The listing builds one solid part. Answer for the finished solid, in the listing's coordinates (mm). Face numbers are marked on the shaded views. A direction names the side the tool comes from. Give positions to 0.01 mm unless a question says otherwise; leave off trailing zeros. Order: outer loops, then holes, each group sorted by start corner. A loop starts at its lowest first (then second) coordinate and runs counter-clockwise, first axis right, second up. Notation, with made-up numbers: (30, -13.75) - (81, -13.75) arc R20 ccw to (81, 20.25) - close; hole circle Ø4 at (4, 14). An arc over 180 degrees is marked (long way). Answer in a Markdown table with one row per item. Add a question column.
```python
from build123d import *

# Parameters (mm, degrees)
BASE_PLATE_SKETCH_W        = 100
BASE_PLATE_SKETCH_H        = 60
BASE_PLATE_100X60X25_DEPTH = 25
T_BLOCK_SKETCH_W           = 70
T_BLOCK_SKETCH_H           = 40
T_BLOCK_70X40X30_DEPTH     = 30
SLOT_15X20_SKETCH_W        = 15
SLOT_15X20_SKETCH_H        = 20
SLOT_15X20_DEPTH_6_DEPTH   = 6
SECOND_SLOT_SKETCH_W       = 15
SECOND_SLOT_SKETCH_H       = 20
SECOND_SLOT_DEPTH_6_DEPTH  = 6
SIDE_ARC_NOTCH_DEPTH       = 60
END_ARC_NOTCH_DEPTH        = 100
BLOCK_RECESS_A_SKETCH_W    = 26
BLOCK_RECESS_A_SKETCH_H    = 5
BLOCK_RECESS_A_DEPTH       = 30
BLOCK_RECESS_B_SKETCH_W    = 26
BLOCK_RECESS_B_SKETCH_H    = 5
BLOCK_RECESS_B_DEPTH       = 30
CROSS_HOLE_SKETCH_R        = 10
CROSS_HOLE_DEPTH           = 55
WEDGE_CUT_A_DEPTH          = 30
WEDGE_FILL_A_DEPTH         = 10
WEDGE_CUT_B_DEPTH          = 30
WEDGE_FILL_B_DEPTH         = 10


with BuildPart() as part:
    # Base Plate Sketch → Base Plate 100x60x25 (new body)
    with BuildSketch(Plane.XY):
        with Locations((50, -30)):
            Rectangle(BASE_PLATE_SKETCH_W, BASE_PLATE_SKETCH_H)
    extrude(amount=BASE_PLATE_100X60X25_DEPTH)

    # T-Block Sketch → T-Block 70x40x30 (add)
    with BuildSketch(Plane.XY.offset(25)):
        with Locations((50, -30)):
            Rectangle(T_BLOCK_SKETCH_W, T_BLOCK_SKETCH_H)
    extrude(amount=T_BLOCK_70X40X30_DEPTH)

    # Slot 15x20 Sketch → Slot 15x20 Depth 6 (cut)
    with BuildSketch(Plane.XY.offset(25)):
        with Locations((7.5, -30)):
            Rectangle(SLOT_15X20_SKETCH_W, SLOT_15X20_SKETCH_H)
    extrude(amount=-SLOT_15X20_DEPTH_6_DEPTH, mode=Mode.SUBTRACT)

    # Second Slot Sketch → Second Slot Depth 6 (cut)
    with BuildSketch(Plane.XY.offset(25)):
        with Locations((92.5, -30)):
            Rectangle(SECOND_SLOT_SKETCH_W, SECOND_SLOT_SKETCH_H)
    extrude(amount=-SECOND_SLOT_DEPTH_6_DEPTH, mode=Mode.SUBTRACT)

    # Side Arc Notch Sketch → Side Arc Notch (cut)
    with BuildSketch(Plane.XZ.offset(60)):
        with BuildLine():
            Line((30, 0), (70, 0))
            ThreePointArc((70, 0), (50, 20), (30, 0))
        make_face()
    extrude(amount=-SIDE_ARC_NOTCH_DEPTH, mode=Mode.SUBTRACT)

    # End Arc Notch Sketch → End Arc Notch (cut)
    with BuildSketch(Plane.ZY):
        with BuildLine():
            Line((0, -15), (0, -45))
            ThreePointArc((0, -45), (15, -30), (0, -15))
        make_face()
    extrude(amount=-END_ARC_NOTCH_DEPTH, mode=Mode.SUBTRACT)

    # Block Recess A Sketch → Block Recess A (cut)
    with BuildSketch(Plane.XY.offset(55)):
        with Locations((50, -12.5)):
            Rectangle(BLOCK_RECESS_A_SKETCH_W, BLOCK_RECESS_A_SKETCH_H)
    extrude(amount=-BLOCK_RECESS_A_DEPTH, mode=Mode.SUBTRACT)

    # Block Recess B Sketch → Block Recess B (cut)
    with BuildSketch(Plane.XY.offset(55)):
        with Locations((50, -47.5)):
            Rectangle(BLOCK_RECESS_B_SKETCH_W, BLOCK_RECESS_B_SKETCH_H)
    extrude(amount=-BLOCK_RECESS_B_DEPTH, mode=Mode.SUBTRACT)

    # Cross Hole Sketch → Cross Hole (cut)
    with BuildSketch(Plane.XY.offset(55)):
        with Locations((50, -30)):
            Circle(CROSS_HOLE_SKETCH_R)
    extrude(amount=-CROSS_HOLE_DEPTH, mode=Mode.SUBTRACT)

    # Wedge Cut A Sketch → Wedge Cut A (cut)
    with BuildSketch(Plane.XZ.offset(50)):
        Polygon((15, 55), (30, 55), (15, 25), align=None)
    extrude(amount=-WEDGE_CUT_A_DEPTH, mode=Mode.SUBTRACT)

    # Wedge Fill A Sketch → Wedge Fill A (add)
    with BuildSketch(Plane.XZ.offset(50)):
        Polygon((15, 25), (15, 55), (30, 55), align=None)
    extrude(amount=-WEDGE_FILL_A_DEPTH)

    # Wedge Cut B Sketch → Wedge Cut B (cut)
    with BuildSketch(Plane.XZ.offset(50)):
        Polygon((85, 55), (70, 55), (85, 25), align=None)
    extrude(amount=-WEDGE_CUT_B_DEPTH, mode=Mode.SUBTRACT)

    # Wedge Fill B Sketch → Wedge Fill B (add)
    with BuildSketch(Plane.XZ.offset(50)):
        Polygon((70, 55), (85, 55), (85, 25), align=None)
    extrude(amount=-WEDGE_FILL_B_DEPTH)


solid = part.part
```
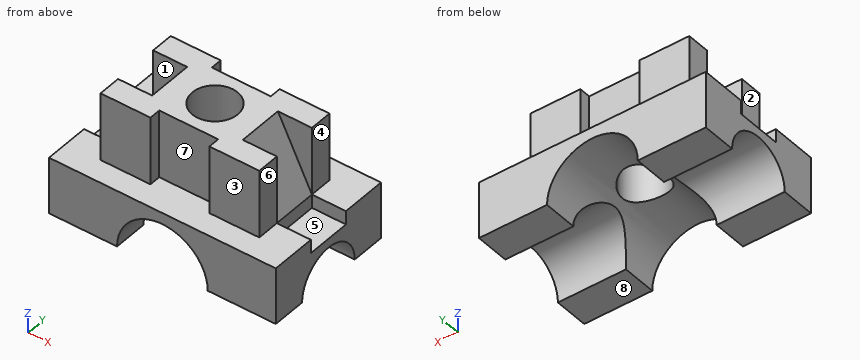
(1) Straight lines are drawn through the part: line 1 (Y direction, x = 16, z = 48); line 2 (X direction, y = -13, z = 44.5); line 3 (Z direction, x = 11, y = -3). For each, find the intervals that lie inside material, in ascending order.
(2) Find section A-A, the plane z = 23. Write down the section's boundary in (x, y).
(3) Find section D-D, the plane z = 3.5. Write down the section's boundary in (x, y), plus the area to 3 significant figures.
(4) The mould has two halves that part along X. Classify the marked faces 6, 7 and 8: +X half, -X half, draft (parallel to the pull), parting line (faces both ways), or undercut.
(5) For the marked faces 1, 2, 3, 4 and 5, determine the directions among +Z, -Z, +X, -X, +Y, -Y from which every point of the face is accessible in a straight line to the end or side of a thin tool.
(6) Find section B-B, the plane x = 50. Write down the section's boundary in (y, z), plus the area to 3 significant figures.
(7) Each of these flat-tipped pins is pushed along its axis until it touches: P1, Ø5.5, axis at y = -12, z = 45, coming from the -X side; P2, Ø6.5, axis at x = 22.5, z = 36.5, coming from the +Y side; P3, Ø4, axis at x = 50, z = 43.5, coming from the +Y side. Where does it stop, or does it pass through?
(8) Find section C-C, the plane y = -30. Write down the section's boundary in (x, z).
Answer key:
| question | item | result |
|---|---|---|
| 1 | line 1 | -50 to -40, -20 to -10 |
| 1 | line 2 | 15 to 37, 63 to 85 |
| 1 | line 3 | 0 to 25 |
| 2 | outline | (0, -60) - (100, -60) - (100, -40) - (85, -40) - (85, -20) - (100, -20) - (100, 0) - (0, 0) - (0, -20) - (15, -20) - (15, -40) - (0, -40) - close; hole circle Ø20 at (50, -30) |
| 3 | outline | (0, -60) - (30.31, -60) - (30.31, -44.59) - (0, -44.59) - close; (0, -15.41) - (30.31, -15.41) - (30.31, 0) - (0, 0) - close; (69.69, -60) - (100, -60) - (100, -44.59) - (69.69, -44.59) - close; (69.69, -15.41) - (100, -15.41) - (100, 0) - (69.69, 0) - close |
| 3 | area | 1,870 mm² |
| 4 | face 6 | +X half |
| 4 | face 7 | undercut |
| 4 | face 8 | draft |
| 5 | face 1 | +Z, -X |
| 5 | face 2 | +Z, -X, +Y, -Y |
| 5 | face 3 | +Z, +X, -X, -Y |
| 5 | face 4 | +Z, +X, +Y, -Y |
| 5 | face 5 | +Z, +X |
| 6 | outline | (-60, 20) - (-40, 20) - (-40, 55) - (-45, 55) - (-45, 25) - (-60, 25) - close; (-20, 20) - (0, 20) - (0, 25) - (-15, 25) - (-15, 55) - (-20, 55) - close |
| 6 | area | 500 mm² |
| 7 | P1 | x = 15 |
| 7 | P2 | y = -10 |
| 7 | P3 | y = -15 |
| 8 | outline | (0, 15) - (36.77, 15) arc R20 cw to (40, 17.32) - (40, 55) - (30, 55) - (15, 25) - (15, 19) - (0, 19) - close; (60, 17.32) arc R20 cw to (63.23, 15) - (100, 15) - (100, 19) - (85, 19) - (85, 25) - (70, 55) - (60, 55) - close |
